Geometry: final body of the model. Coordinates: model frame, mm. Face numbers are marked on the shaded views. Round coordinates to 2 decimals unless told otherwise and drop trailing zeros. Loops run counter-clockwise (first coordinate to the right, second up) from the corner with the lowest first, then second, coordinate; pieces in that order, holes last. Notation, with made-up numbers: (3, -22) -> (23, -22) arc R25 cw to (23, 7) -> close; hole circle Ø8 at (-6, 87.25). An arc over 180 degrees is marked (long way). Answer in a Markdown table with one row per item.
```python
from build123d import *

# Parameters (mm, degrees)
CYLINDER_PROFILE_28_R           = 14
CYLINDER_BODY_28X24_DEPTH       = 24
HOLE_CIRCLE_SKETCH_3X_6_PCD16_R = 3
THROUGH_HOLES_3X_6_PCD16_DEPTH  = 29
CENTRE_HOLE_SKETCH_6_R          = 3
CENTRE_HOLE_6_DEPTH             = 29


with BuildPart() as part:
    # Cylinder Profile Ø28 → Cylinder Body Ø28x24 (new body)
    with BuildSketch(Plane(origin=(0, 0, 0), x_dir=(1, 0, 0), z_dir=(0, 1, 0))):
        with Locations(Location((0, 0, 0), (0, 0, 270))):
            Circle(CYLINDER_PROFILE_28_R)
    extrude(amount=CYLINDER_BODY_28X24_DEPTH)

    # Hole Circle Sketch 3xØ6 PCD16 → Through Holes 3xØ6 PCD16 (cut)
    with BuildSketch(Plane(origin=(0, 24, 0), x_dir=(1, 0, 0), z_dir=(0, 1, 0))):
        with Locations(Location((0, 8, 0), (0, 0, 270))):
            Circle(HOLE_CIRCLE_SKETCH_3X_6_PCD16_R)
        with Locations(Location((6.92820323, -4, 0), (0, 0, 270))):
            Circle(HOLE_CIRCLE_SKETCH_3X_6_PCD16_R)
        with Locations(Location((-6.92820323, -4, 0), (0, 0, 270))):
            Circle(HOLE_CIRCLE_SKETCH_3X_6_PCD16_R)
    extrude(amount=-THROUGH_HOLES_3X_6_PCD16_DEPTH, mode=Mode.SUBTRACT)

    # Centre Hole Sketch Ø6 → Centre Hole Ø6 (cut)
    with BuildSketch(Plane(origin=(0, 24, 0), x_dir=(1, 0, 0), z_dir=(0, 1, 0))):
        with Locations(Location((0, 0, 0), (0, 0, 270))):
            Circle(CENTRE_HOLE_SKETCH_6_R)
    extrude(amount=-CENTRE_HOLE_6_DEPTH, mode=Mode.SUBTRACT)


solid = part.part
```
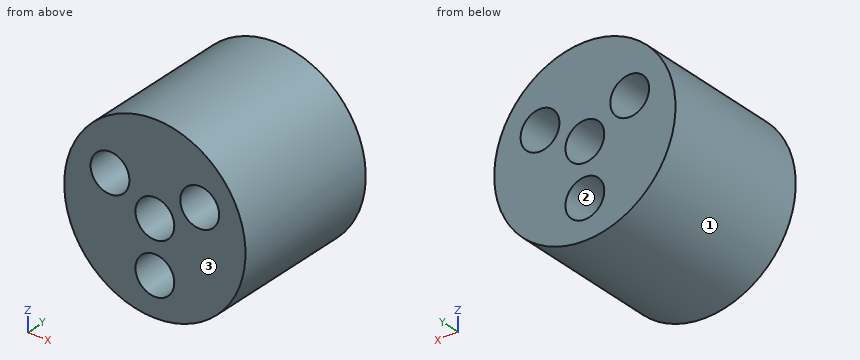
Item 1: Line query: probe 1 along X at (y, z) = (6.5, 0); probe 2 along Z at (x, y) = (-0.25, 17.75); probe 3 along Z at (x, y) = (-1.5, 4.5). Output: solid intervals per line, ascending. Write a range as [from, to].
Answer:
| item | result |
|---|---|
| probe 1 | x = [-14, -3], [3, 14] |
| probe 2 | z = [-14, -10.99], [-5.01, -2.99], [2.99, 14] |
| probe 3 | z = [-13.92, -10.6], [-5.4, -2.6], [2.6, 13.92] |
Item 2: Cut plane D-D (x = 1.25). Output: boundary loops of the cut face in (y, z).
Answer:
| item | result |
|---|---|
| outline | (0, -13.94) -> (24, -13.94) -> (24, -10.73) -> (0, -10.73) -> close; (0, -5.27) -> (24, -5.27) -> (24, -2.73) -> (0, -2.73) -> close; (0, 2.73) -> (24, 2.73) -> (24, 13.94) -> (0, 13.94) -> close |
Item 3: Cut plane A-A (z = 0). Output: boundary loops of the cut face in (x, y), then the cut area to 3 significant figures.
Answer:
| item | result |
|---|---|
| outline | (-14, 0) -> (-3, 0) -> (-3, 24) -> (-14, 24) -> close; (3, 0) -> (14, 0) -> (14, 24) -> (3, 24) -> close |
| area | 528 mm² |
Item 4: Draft query along Z for the marked faces 1, 2 and 3. Return one class per face: pulls with the +Z half, pulls with the -Z half, needs draft (parallel to the pull), parting line crosses it, or undercut.
Answer:
| item | result |
|---|---|
| face 1 | parting line crosses it |
| face 2 | undercut |
| face 3 | needs draft |
Item 5: Pin query (flat end, axial travel): pin 1 Ø2 at (y, z) = (8, -10.5) entering from +X; pin 2 Ø2 at (x, y) = (-2.5, 13) entering from +Z; pin 3 Ø1.5 at (x, y) = (-6, 6) entering from -Z. Return the tip coordinate at first contact, or that it passes through.
Answer:
| item | result |
|---|---|
| pin 1 | stops at x = 10.28 |
| pin 2 | stops at z = 13.92 |
| pin 3 | stops at z = -12.98 |
Item 6: Cut plane B-B (x = -8). Output: boundary loops of the cut face in (y, z).
Answer:
| item | result |
|---|---|
| outline | (0, -11.49) -> (24, -11.49) -> (24, 1.2) -> (0, 1.2) -> close; (0, 6.8) -> (24, 6.8) -> (24, 11.49) -> (0, 11.49) -> close |
Item 7: Cut plane C-C (z = 4). Output: boundary loops of the cut face in (x, y), then the cut area to 3 significant figures.
Answer:
| item | result |
|---|---|
| outline | (-13.42, 0) -> (-9.93, 0) -> (-9.93, 24) -> (-13.42, 24) -> close; (-3.93, 0) -> (3.93, 0) -> (3.93, 24) -> (-3.93, 24) -> close; (9.93, 0) -> (13.42, 0) -> (13.42, 24) -> (9.93, 24) -> close |
| area | 356 mm² |
